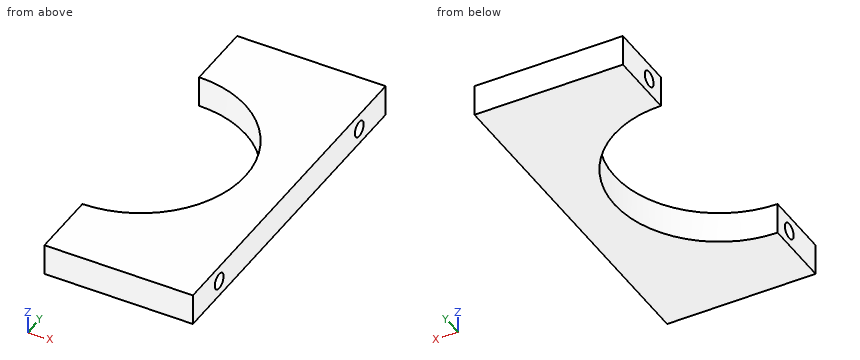
from build123d import *

# Parameters (mm, degrees)
BOSS_EXTRUDE1_DEPTH = 3
SKETCH3_R           = 0.75
CUT_EXTRUDE1_DEPTH  = 31.209452006


with BuildPart() as part:
    # Sketch2 → Boss-Extrude1 (new body)
    with BuildSketch(Plane.XY):
        with BuildLine():
            Line((16.5, -26.504131531), (30.682454029, -26.504131531))
            Line((30.682454029, -26.504131531), (30.682454029, 6.495868469))
            Line((30.682454029, 6.495868469), (16.5, 6.495868469))
            Line((16.5, 6.495868469), (16.5, -0.004131531))
            ThreePointArc((16.5, -0.004131531), (26.5, -10.004131531), (16.5, -20.004131531))
            Line((16.5, -20.004131531), (16.5, -26.504131531))
        make_face()
    extrude(amount=-BOSS_EXTRUDE1_DEPTH)

    # Sketch3 → Cut-Extrude1 (cut, through all)
    with BuildSketch(Plane(origin=(30.682454029, 0, 0), x_dir=(0, 0, -1), z_dir=(1, 0, 0))):
        with Locations((1.5, -22.004131531)):
            Circle(SKETCH3_R)
        with Locations(Location((1.5, 1.995868469, 0), (0, 0, 180))):
            Circle(SKETCH3_R)
    extrude(amount=-CUT_EXTRUDE1_DEPTH, mode=Mode.SUBTRACT)


solid = part.part
Here's how the part is built. I have some questions about the finished solid (model axes, mm). Round coordinates to 2 decimals unless told otherwise and drop trailing zeros. Order: outer loops, then holes, each group sorted by start corner. A loop starts at its lowest first (then second) coordinate and runs counter-clockwise, first axis right, second up. Notation, with made-up numbers: M -23.5,70.5 L 15.5,70.5 A23 ccw 15.5,106.5 Z; hole C -3.75,18.25 d7. An arc over 180 degrees is marked long. Return JSON: item names as keys, results as strings. Group by question number.
1. If we section it at A-A on z = -1.5: List the corners of the cut face in (x, y) for me, then the cut area to 3 significant figures.
2. If we section it at D-D on y = -11: List the corners of the cut face in (x, z) for me.
3. If we section it at C-C on x = 17.75: List the corners of the cut face in (y, z) for me, then the cut area to 3 significant figures.
4. If we section it at B-B on x = 25.75: List the corners of the cut face in (y, z) for me, then the cut area to 3 significant figures.
5. Please list where these lines run through material, in increasing order: probe 1 along Y at (x, z) = (27, -1.5); probe 2 along Z at (x, y) = (18.5, -22); probe 3 along Y at (x, z) = (21.25, -1.5).
Reply:
{
 "1": {"outline": "M 16.5,-26.5 L 30.68,-26.5 L 30.68,-22.75 L 16.5,-22.75 Z; M 16.5,-21.25 L 30.68,-21.25 L 30.68,1.25 L 16.5,1.25 L 16.5,0 A10 cw 16.5,-20 Z; M 16.5,2.75 L 30.68,2.75 L 30.68,6.5 L 16.5,6.5 Z", "area": "268 mm^2"},
 "2": {"outline": "M 26.45,-3 L 30.68,-3 L 30.68,0 L 26.45,0 Z"},
 "3": {"outline": "M -26.5,-3 L -19.93,-3 L -19.93,0 L -26.5,0 Z; M -0.08,-3 L 6.5,-3 L 6.5,0 L -0.08,0 Z; hole C -22,-1.5 d1.5; hole C 2,-1.5 d1.5", "area": "35.9 mm^2"},
 "4": {"outline": "M -26.5,-3 L -13.8,-3 L -13.8,0 L -26.5,0 Z; M -6.2,-3 L 6.5,-3 L 6.5,0 L -6.2,0 Z; hole C -22,-1.5 d1.5; hole C 2,-1.5 d1.5", "area": "72.7 mm^2"},
 "5": {"probe 1": "-26.5 to -22.75, -21.25 to 1.25, 2.75 to 6.5", "probe 2": "-3 to -2.25, -0.75 to 0", "probe 3": "-26.5 to -22.75, -21.25 to -18.8, -1.2 to 1.25, 2.75 to 6.5"}
}
